Could you check a few things on this model? Use its own coordinates, in mm. Face numbers are marked on the shaded views. A direction names the side the tool comes from. Round coordinates to 2 decimals unless told otherwise and drop trailing zeros. Loops run counter-clockwise (first coordinate to the right, second up) from the corner with the lowest first, then second, coordinate; pieces in that order, holes last. Notation, with made-up numbers: (-36, -1.5) -> (-20, -1.5) arc R14 ccw to (-20, 16.5) -> close; hole circle Ø8 at (88.25, 28.5). An arc over 180 degrees is marked (long way). Write each question's results on one line, items separated by ' | '. Start each with the question number.
1) Imagine slicing it at C-C, the plane y = 40.5. List the corners of the cut face in (x, z) for me.
2) We'd pull the mould along X, two halves only. Please class the marked faces 1, 2 and 3: pulls with the +X half, pulls with the -X half, needs draft (parallel to the pull), parting line crosses it, or undercut.
3) If I drill on probe 1 along Y at (x, z) = (-43, -14.5); probe 2 along X at (y, z) = (120, -11.5); probe 3 along Z at (x, y) = (-17.5, 137), over which ranges is the centre line in solid material (lowest first)?
4) Which directions (+Z, -Z, +X, -X, +Y, -Y) give clear straight access to the entire face, cutting with the end or side of a thin tool? Please do the marked faces 4 and 5.
5) Imagine slicing it at B-B, the plane z = -16. List the corners of the cut face in (x, y) for me, plus the area to 3 significant figures.
6) Imagine slicing it at A-A, the plane x = 83. List the corners of the cut face in (y, z) for me, plus the area to 3 significant figures.
7) For P1, Ø6, axis at x = -119.5, y = 75.5, coming from the -Z side, with a flat end and sliding along its axis, tell me the tip position at first contact or that it passes through.
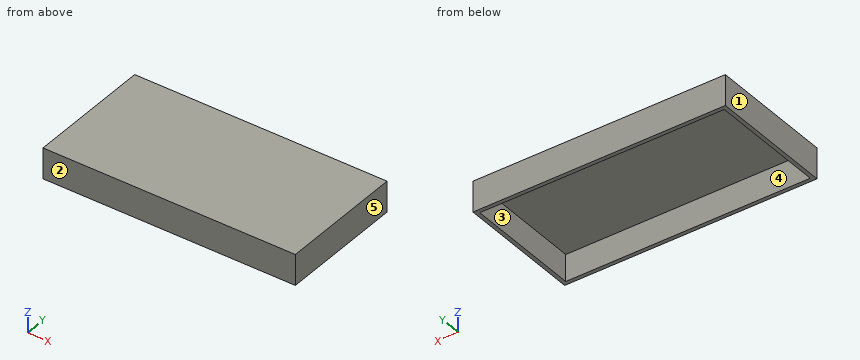
from build123d import *

# Parameters (mm, degrees)
SKETCH1_W           = 390
SKETCH1_H           = 47.5
BOSS_EXTRUDE1_DEPTH = 195
SHELL1_T            = -6


with BuildPart() as part:
    # Sketch1 → Boss-Extrude1 (new body)
    with BuildSketch(Plane(origin=(0, 0, 0), x_dir=(1, 0, 0), z_dir=(0, 1, 0))):
        Rectangle(SKETCH1_W, SKETCH1_H)
    extrude(amount=BOSS_EXTRUDE1_DEPTH)

    # Shell1
    shell1_openings = [part.faces().sort_by_distance(p)[0] for p in [
        (0, 97.5, -23.75),
    ]]
    offset(amount=SHELL1_T, openings=shell1_openings, kind=Kind.INTERSECTION)


solid = part.part
Checked values:
1) outline: (-195, -23.75) -> (-189, -23.75) -> (-189, 17.75) -> (189, 17.75) -> (189, -23.75) -> (195, -23.75) -> (195, 23.75) -> (-195, 23.75) -> close
2) face 1: pulls with the -X half | face 2: needs draft | face 3: undercut
3) probe 1: 0 to 6, 189 to 195 | probe 2: -195 to -189, 189 to 195 | probe 3: 17.75 to 23.75
4) face 4: -Z | face 5: +Z, -Z, +X, +Y, -Y
5) outline: (-195, 0) -> (195, 0) -> (195, 195) -> (-195, 195) -> close; hole (-189, 6) -> (189, 6) -> (189, 189) -> (-189, 189) -> close | area: 6,880 mm^2
6) outline: (0, -23.75) -> (6, -23.75) -> (6, 17.75) -> (189, 17.75) -> (189, -23.75) -> (195, -23.75) -> (195, 23.75) -> (0, 23.75) -> close | area: 1,670 mm^2
7) P1: z = 17.75
